Build history of the part. All positions in model axes, mm. A direction names the side the tool comes from. Give positions to 0.01 mm unless a question says otherwise; leave off trailing zeros. Order: outer loops, then holes, each group sorted by start corner. A loop starts at its lowest first (then second) coordinate and runs counter-clockwise, first axis right, second up. Notation, with made-up numbers: (47, -19) - (54, -19) arc R21 cw to (54, -2) - close; hole circle Ø1 at (51.5, 39.25). An arc over 180 degrees is marked (long way). Use a Markdown table: item, result. Add a question column.
(1) Flat gauge pins, fed straight in: pin 1 (4 mm diameter, centred on x = 10.5, y = 5.5, fed in from +Z); pin 2 (2 mm diameter, centred on x = 16.5, y = -1, fed in from -Z); pin 3 (1 mm diameter, centred on x = 9, z = -5.5, fed in from -Y). Where does each tip first touch, or does it go through?
(2) Which spindle directions (+Z, -Z, +X, -X, +Y, -Y) get a long thin tool onto all of the face, cutting with end or side? Do faces 4 (the face through (9.204, 0.33, 7.493)), 5 (the face through (13, 2, 5)), 6 (the face through (3.21, -4.88, 1.08)). Say none if no direction does.
(3) Wall check: line 1 (X direction, y = 4.5, z = -2.75); line 2 (Z direction, x = 14, y = 0.25); line 3 (Y direction, x = 22, z = 0). Give the ranges that are in metal, low to high.
(4) Slice it at A-A (z = 0). Write the cut outline in (x, y).
(5) Slice it at C-C (x = 4.75). Write the cut outline in (y, z).
(6) Mould opens along X. For faces 1 (the face through (21.54, 3.92, -2.5)), 2 (the face through (22.79, -4.88, 1.08)), 3 (the face through (24, 0, 0)) say: +X half, -X half, draft (parallel to the pull), parting line (faces both ways), or undercut.
from build123d import *

# Parameters (mm, degrees)
SKETCH_1_R      = 5
EXTRUDE_1_DEPTH = 6
CHAMFER_1_SIZE  = 0.5
SKETCH_2_R      = 7.5
EXTRUDE_2_DEPTH = 7
CHAMFER_2_SIZE  = 0.5
SKETCH_3_R      = 5
EXTRUDE_3_DEPTH = 8
SKETCH_4_R      = 4.65
EXTRUDE_4_DEPTH = 1.1
SKETCH_5_R      = 5
EXTRUDE_5_DEPTH = 1.9
CHAMFER_3_SIZE  = 0.5


with BuildPart() as part:
    # 草图1 → 凸台-拉伸1 (new body)
    with BuildSketch(Plane(origin=(0, 0, 0), x_dir=(0, 0, -1), z_dir=(1, 0, 0))):
        Circle(SKETCH_1_R)
    extrude(amount=EXTRUDE_1_DEPTH)

    # 倒角1
    chamfer_1_edges = [part.edges().sort_by_distance(p)[0] for p in [
        (0, 0, 5),
    ]]
    chamfer(chamfer_1_edges, length=CHAMFER_1_SIZE)

    # 草图2 → 凸台-拉伸2 (add)
    with BuildSketch(Plane(origin=(6, 0, 0), x_dir=(0, 0, -1), z_dir=(1, 0, 0))):
        Circle(SKETCH_2_R)
    extrude(amount=EXTRUDE_2_DEPTH)

    # 倒角2
    chamfer_2_edges = [part.edges().sort_by_distance(p)[0] for p in [
        (13, 0, 7.5),
    ]]
    chamfer(chamfer_2_edges, length=CHAMFER_2_SIZE)

    # 草图3 → 凸台-拉伸3 (add)
    with BuildSketch(Plane(origin=(13, 0, 0), x_dir=(0, 0, -1), z_dir=(1, 0, 0))):
        Circle(SKETCH_3_R)
    extrude(amount=EXTRUDE_3_DEPTH)

    # 草图4 → 凸台-拉伸4 (add)
    with BuildSketch(Plane(origin=(21, 0, 0), x_dir=(0, 0, -1), z_dir=(1, 0, 0))):
        Circle(SKETCH_4_R)
    extrude(amount=EXTRUDE_4_DEPTH)

    # 草图5 → 凸台-拉伸5 (add)
    with BuildSketch(Plane(origin=(22.1, 0, 0), x_dir=(0, 0, -1), z_dir=(1, 0, 0))):
        Circle(SKETCH_5_R)
    extrude(amount=EXTRUDE_5_DEPTH)

    # 倒角3
    chamfer_3_edges = [part.edges().sort_by_distance(p)[0] for p in [
        (24, 0, 5),
    ]]
    chamfer(chamfer_3_edges, length=CHAMFER_3_SIZE)


solid = part.part
Solution:
| question | item | result |
|---|---|---|
| 1 | pin 1 | z = 6.63 |
| 1 | pin 2 | z = -5 |
| 1 | pin 3 | y = -5.59 |
| 2 | face 4 | +X, -X |
| 2 | face 5 | +X |
| 2 | face 6 | -X |
| 3 | line 1 | 6 to 13 |
| 3 | line 2 | -4.99 to 4.99 |
| 3 | line 3 | -4.65 to 4.65 |
| 4 | outline | (0, -4.5) - (0.5, -5) - (6, -5) - (6, -7.5) - (12.5, -7.5) - (13, -7) - (13, -5) - (21, -5) - (21, -4.65) - (22.1, -4.65) - (22.1, -5) - (23.5, -5) - (24, -4.5) - (24, 4.5) - (23.5, 5) - (22.1, 5) - (22.1, 4.65) - (21, 4.65) - (21, 5) - (13, 5) - (13, 7) - (12.5, 7.5) - (6, 7.5) - (6, 5) - (0.5, 5) - (0, 4.5) - close |
| 5 | outline | circle Ø10 at (0, 0) |
| 6 | face 1 | undercut |
| 6 | face 2 | draft |
| 6 | face 3 | +X half |
